Here's how the part is built. I have some questions about the finished solid (model axes, mm). A direction names the side the tool comes from. Round coordinates to 2 decimals unless told otherwise and drop trailing zeros. Write each loop counter-clockwise with the first axis right and the second up, starting at its lowest first coordinate (ties: lowest second). Pieces come first, ordered by that corner, then holes. Notation, with made-up numbers: (-0.75, 9.5) - (3.25, 9.5) arc R25 cw to (3.25, 28.5) - close; hole circle Ø6 at (-31.5, 76.5). An arc over 180 degrees is marked (long way). One line per question, with ' | ' between items. Start each with the question number.
(1) Imagine slicing it at A-A (x = -7). Write out the boundary of the cut face in (y, z), plus the area to 3 significant figures.
(2) Thinking about a two-plate mould opening in Y: for faces 4 (the flat face through (-4, 7, 30)), 5 (the cylindrical face through (-14, 97, 0)), 6 (the flat face through (14, 65, 0)), which applies, pulls with the +Y half, pulls with the -Y half, needs draft (parallel to the pull), parting line crosses it, or undercut?
(3) Imagine slicing it at D-D (z = -14). Write out the boundary of the cut face in (x, y), plus the area to 3 significant figures.
(4) For faces 1 (the flat face through (4, 7, -30)), 2 (the flat face through (11, 68, 0)), 3 (the flat face through (4, 7, 30)), which set-ups out of +Z, -Z, +X, -X, +Y, -Y let a thin tool reach every point of the face, with its end or its side?
(5) If I drill on L1, parallel to Y at x = -15, z = 0; L2, parallel to Z at x = 14.5, y = 85; L3, parallel to X at y = 26, z = -11.5, over which ranges is the centre line in solid material (lowest first)?
(6) Will these pins go through, and if not, where does the flat tip stop? pin 1 (12 mm diameter, centred on x = 10, z = -17, fed in from +Y); pin 2 (6 mm diameter, centred on x = -12, y = 70.5, fed in from -Z); pin 3 (2.5 mm diameter, centred on x = -30.5, y = 5.5, fed in from +Z); pin 4 (23.5 mm diameter, centred on x = 0, z = 0, fed in from +Y).
(7) Imagine slicing it at C-C (y = 60.5). Write out the boundary of the cut face in (x, z), plus the area to 3 significant figures.
(8) Imagine slicing it at B-B (z = -29). Write out the boundary of the cut face in (x, y), plus the area to 3 significant figures.
from build123d import *
from build123d.topology import SkipClean

# Parameters (mm, degrees)
BASE_FLANGE_DEPTH       = 15
CENTRE_HOLE_SKETCH_R    = 9
CENTRE_HOLE_18_DEPTH    = 15
LUG_START               = 10
LUG_BASE_PAD_DEPTH      = 10
CLEVIS_LUG_BLOCKS_DEPTH = 70
LUG_PROFILE_CUT_DEPTH   = 54
LUG_EYE_BOSS_DEPTH      = 5.5
LUG_START_2             = -5.5
LUG_WEB_DEPTH           = 5.5


with BuildPart() as part:
    # Base Flange Sketch → Base Flange (new body)
    with BuildSketch(Plane(origin=(0, 0, 0), x_dir=(1, 0, 0), z_dir=(0, 1, 0))):
        with BuildLine():
            ThreePointArc((26, -4), (25.846039759, -3.997035932), (25.692307692, -3.988148122))
            ThreePointArc((25.692307692, -3.988148122), (18.384776311, -18.384776311), (3.988148122, -25.692307692))
            ThreePointArc((3.988148122, -25.692307692), (3.997035932, -25.846039759), (4, -26))
            Line((4, -26), (4, -33.763886032))
            ThreePointArc((4, -33.763886032), (24.04163056, -24.04163056), (33.763886032, -4))
            Line((33.763886032, -4), (26, -4))
        make_face()
        with BuildLine():
            ThreePointArc((25.692307692, 3.988148122), (25.846039759, 3.997035932), (26, 4))
            Line((26, 4), (33.763886032, 4))
            ThreePointArc((33.763886032, 4), (24.04163056, 24.04163056), (4, 33.763886032))
            Line((4, 33.763886032), (4, 26))
            ThreePointArc((4, 26), (3.997035932, 25.846039759), (3.988148122, 25.692307692))
            ThreePointArc((3.988148122, 25.692307692), (18.384776311, 18.384776311), (25.692307692, 3.988148122))
        make_face()
        with BuildLine():
            ThreePointArc((-25.692307692, 3.988148122), (-18.384776311, 18.384776311), (-3.988148122, 25.692307692))
            ThreePointArc((-3.988148122, 25.692307692), (-3.997035932, 25.846039759), (-4, 26))
            Line((-4, 26), (-4, 33.763886032))
            ThreePointArc((-4, 33.763886032), (-24.04163056, 24.04163056), (-33.763886032, 4))
            Line((-33.763886032, 4), (-26, 4))
            ThreePointArc((-26, 4), (-25.846039759, 3.997035932), (-25.692307692, 3.988148122))
        make_face()
        with BuildLine():
            ThreePointArc((-4, -26), (-3.997035932, -25.846039759), (-3.988148122, -25.692307692))
            ThreePointArc((-3.988148122, -25.692307692), (-18.384776311, -18.384776311), (-25.692307692, -3.988148122))
            ThreePointArc((-25.692307692, -3.988148122), (-25.846039759, -3.997035932), (-26, -4))
            Line((-26, -4), (-33.763886032, -4))
            ThreePointArc((-33.763886032, -4), (-24.04163056, -24.04163056), (-4, -33.763886032))
            Line((-4, -33.763886032), (-4, -26))
        make_face()
        with BuildLine():
            ThreePointArc((25.692307692, -3.988148122), (22, 0), (25.692307692, 3.988148122))
            ThreePointArc((25.692307692, 3.988148122), (18.384776311, 18.384776311), (3.988148122, 25.692307692))
            ThreePointArc((3.988148122, 25.692307692), (0, 22), (-3.988148122, 25.692307692))
            ThreePointArc((-3.988148122, 25.692307692), (-18.384776311, 18.384776311), (-25.692307692, 3.988148122))
            ThreePointArc((-25.692307692, 3.988148122), (-22, 0), (-25.692307692, -3.988148122))
            ThreePointArc((-25.692307692, -3.988148122), (-18.384776311, -18.384776311), (-3.988148122, -25.692307692))
            ThreePointArc((-3.988148122, -25.692307692), (0, -22), (3.988148122, -25.692307692))
            ThreePointArc((3.988148122, -25.692307692), (18.384776311, -18.384776311), (25.692307692, -3.988148122))
        make_face()
    extrude(amount=BASE_FLANGE_DEPTH)

    # Centre Hole Sketch → Centre Hole _18 (cut)
    with BuildSketch(Plane(origin=(0, 15, 0), x_dir=(1, 0, 0), z_dir=(0, 1, 0))):
        with Locations(Location((0, 0, 0), (0, 0, 270))):
            Circle(CENTRE_HOLE_SKETCH_R)
    extrude(amount=-CENTRE_HOLE_18_DEPTH, mode=Mode.SUBTRACT)

    # Lug Base Sketch → Lug Base Pad (add)
    with BuildSketch(Plane(origin=(0, 15, 0), x_dir=(1, 0, 0), z_dir=(0, 1, 0)).offset(LUG_START)):
        Polygon((11, -11), (0, -11), (-11, -11), (-11, -16.5), (11, -16.5), align=None)
        Polygon((0, 11), (11, 11), (11, 16.5), (-11, 16.5), (-11, 11), align=None)
        with BuildLine():
            Line((0, -9), (0, -11))
            Line((0, -11), (11, -11))
            Line((11, -11), (11, 11))
            Line((11, 11), (0, 11))
            Line((0, 11), (0, 9))
            ThreePointArc((0, 9), (6.363961031, 6.363961031), (9, 0))
            ThreePointArc((9, 0), (6.363961031, -6.363961031), (0, -9))
        make_face()
        with BuildLine():
            Line((-11, -11), (0, -11))
            Line((0, -11), (0, -9))
            ThreePointArc((0, -9), (-9, 0), (0, 9))
            Line((0, 9), (0, 11))
            Line((0, 11), (-11, 11))
            Line((-11, 11), (-11, -11))
        make_face()
    extrude(amount=-LUG_BASE_PAD_DEPTH)

    # Sketch3_3 → Clevis Lug Blocks (add)
    with BuildSketch(Plane(origin=(0, 15, 0), x_dir=(1, 0, 0), z_dir=(0, 1, 0))):
        Polygon((11, 11), (11, -11), (11, -16.5), (16.5, -16.5), (16.5, 16.5), (11, 16.5), align=None)
        Polygon((-11, -16.5), (-11, -11), (-11, 11), (-11, 16.5), (-16.5, 16.5), (-16.5, -16.5), align=None)
    extrude(amount=CLEVIS_LUG_BLOCKS_DEPTH)

    # Lug Profile Sketch → Lug Profile Cut (cut)
    with BuildSketch(Plane(origin=(16.5, 0, 0), x_dir=(0, 0, -1), z_dir=(1, 0, 0))):
        Polygon((16.5, 85), (12, 85), (16.5, 45), align=None)
        Polygon((-16.5, 45), (-12, 85), (-16.5, 85), align=None)
        Polygon((-11, 30), (-11, 45), (-7.5, 65), (0, 65), (7.5, 65), (11, 45), (11, 30), align=None)
        with BuildLine():
            Line((7.5, 85), (-7.5, 85))
            ThreePointArc((-7.5, 85), (0, 77.5), (7.5, 85))
        make_face()
        with BuildLine():
            ThreePointArc((7.5, 85), (0, 92.5), (-7.5, 85))
            Line((-7.5, 85), (7.5, 85))
        make_face()
    extrude(amount=-LUG_PROFILE_CUT_DEPTH, mode=Mode.SUBTRACT)

    # Sketch6_4 → Lug Eye Boss (add)
    with SkipClean():  # the faces are left unmerged after this step: merging them gives an invalid solid
        with BuildSketch(Plane(origin=(16.5, 0, 0), x_dir=(0, 0, -1), z_dir=(1, 0, 0))):
            with BuildLine():
                Line((-7.5, 85), (-12, 85))
                ThreePointArc((-12, 85), (0, 73), (12, 85))
                Line((12, 85), (7.5, 85))
                ThreePointArc((7.5, 85), (0, 77.5), (-7.5, 85))
            make_face()
            with BuildLine():
                ThreePointArc((12, 85), (0, 97), (-12, 85))
                Line((-12, 85), (-7.5, 85))
                ThreePointArc((-7.5, 85), (0, 92.5), (7.5, 85))
                Line((7.5, 85), (12, 85))
            make_face()
        extrude(amount=-LUG_EYE_BOSS_DEPTH)

    # Lug Web Sketch → Lug Web (add)
    with SkipClean():  # the faces are left unmerged after this step: merging them gives an invalid solid
        with BuildSketch(Plane.ZY.offset(16.5).offset(LUG_START_2)):
            with BuildLine():
                Line((7.5, 85), (12, 85))
                ThreePointArc((12, 85), (0, 97), (-12, 85))
                Line((-12, 85), (-7.5, 85))
                ThreePointArc((-7.5, 85), (0, 92.5), (7.5, 85))
            make_face()
        extrude(amount=LUG_WEB_DEPTH)


solid = part.part
Check sheet entries:
1) outline: (0, -33.27) - (15, -33.27) - (15, -16.5) - (25, -16.5) - (25, -5.66) - (0, -5.66) - close; (0, 5.66) - (25, 5.66) - (25, 16.5) - (15, 16.5) - (15, 33.27) - (0, 33.27) - close | area: 1,050 mm^2
2) face 4: needs draft | face 5: pulls with the +Y half | face 6: undercut
3) outline: (-30.98, 0) - (30.98, 0) - (30.98, 15) - (16.5, 15) - (16.5, 67.22) - (11, 67.22) - (11, 25) - (-11, 25) - (-11, 67.22) - (-16.5, 67.22) - (-16.5, 15) - (-30.98, 15) - close | area: 1,720 mm^2
4) face 1: -Z, +Y, -Y | face 2: +Z, -Z, +Y | face 3: +Z, +Y, -Y
5) L1: 0 to 30, 65 to 77.5, 92.5 to 97 | L2: -12 to -7.5, 7.5 to 12 | L3: -16.5 to -11, 11 to 16.5
6) pin 1: y = 89.6 | pin 2: z = -13.97 | pin 3: z = 17.33 | pin 4: y = 97
7) outline: (-16.5, -14.76) - (-11, -14.76) - (-11, -8.29) - (-16.5, -8.29) - close; (-16.5, 8.29) - (-11, 8.29) - (-11, 14.76) - (-16.5, 14.76) - close; (11, -14.76) - (16.5, -14.76) - (16.5, -8.29) - (11, -8.29) - close; (11, 8.29) - (16.5, 8.29) - (16.5, 14.76) - (11, 14.76) - close | area: 142 mm^2
8) outline: (-17.75, 0) - (-4, 0) - (-4, 15) - (-17.75, 15) - close; (4, 0) - (17.75, 0) - (17.75, 15) - (4, 15) - close | area: 412 mm^2
